Geometry: final body of the model. Coordinates: model frame, mm. A direction names the side the tool comes from. Round coordinates to 2 decimals unless told otherwise and drop trailing zeros. Write each loop counter-clockwise with the first axis right and the second up, starting at its lowest first coordinate (ties: lowest second). Pieces come first, ordered by that corner, then holes. Notation, with made-up numbers: (34.5, 44.5) - (69.5, 44.5) arc R20 cw to (69.5, 51.5) - close; hole circle Ø9 at (37, -10). An arc over 180 degrees is marked (long way). Write each question's results on one line, items separated by ' | '.
from build123d import *
from build123d.topology import SkipClean

# Parameters (mm, degrees)
BASE_DISC_SKETCH_R         = 31
BASE_DISC_DEPTH            = 13
BASE_SLOT_SKETCH_3X_R      = 3
BASE_SLOTS_3X_DEPTH        = 6
CLAMP_START                = -24
CLAMP_LUG_DEPTH            = 24
LUG_HOLE_A_SKETCH_R        = 4.680098696
LUG_HOLE_A_DEPTH           = 57.727418415
LUG_HOLE_B_SKETCH_R        = 5.830404683
LUG_HOLE_B_DEPTH           = 59.693575035
CLAMP_LUG_PATTERN_3X_COUNT = 3
FACE_RECESS_SKETCH_R       = 10
FACE_RECESS_2MM_DEPTH      = 2
LUG_CHAMFER_5MM_SIZE       = 5


with BuildPart() as part:
    # Base Disc Sketch → Base Disc (new body)
    with BuildSketch(Plane.XY):
        with Locations(Location((0, 0, 0), (0, 0, 180))):
            Circle(BASE_DISC_SKETCH_R)
    extrude(amount=BASE_DISC_DEPTH)

    # Base Slot Sketch 3x → Base Slots 3x (cut)
    with BuildSketch(Plane.XY):
        with Locations((-6.470476128, -24.148145657)):
            Circle(BASE_SLOT_SKETCH_3X_R)
        with Locations((-17.67766953, 17.67766953)):
            Circle(BASE_SLOT_SKETCH_3X_R)
        with Locations((24.148145657, 6.470476128)):
            Circle(BASE_SLOT_SKETCH_3X_R)
    extrude(amount=BASE_SLOTS_3X_DEPTH, mode=Mode.SUBTRACT)

    # Clamp Lug Sketch → Clamp Lug (add)
    with SkipClean():  # the faces are left unmerged after this step: merging them gives an invalid solid
        with BuildSketch(Plane.XY.offset(CLAMP_START)):
            with BuildLine():
                Line((5, 8.660254038), (5, 30.594117082))
                ThreePointArc((5, 30.594117082), (7.526051267, 30.072554802), (10, 29.342801502))
                Line((10, 29.342801502), (10, 8.306623863))
                ThreePointArc((10, 8.306623863), (10.309933784, 5.952443046), (12.193747285, 4.506942106))
                Line((12.193747285, 4.506942106), (30.411611519, -6.011146713))
                ThreePointArc((30.411611519, -6.011146713), (29.806622049, -8.518525814), (28.995282599, -10.966931522))
                Line((28.995282599, -10.966931522), (10, 0))
                ThreePointArc((10, 0), (8.660254038, 5), (5, 8.660254038))
            make_face()
        clamp_lug = extrude(amount=CLAMP_LUG_DEPTH)

    # Lug Hole A Sketch → Lug Hole A (cut, through all)
    with SkipClean():  # the faces are left unmerged after this step: merging them gives an invalid solid
        with BuildSketch(Plane(origin=(10, 0, 0), x_dir=(0, 0, -1), z_dir=(1, 0, 0))):
            with Locations(Location((14, 19.342801502, 0), (0, 0, 90))):
                Circle(LUG_HOLE_A_SKETCH_R)
        lug_hole_a = extrude(amount=-LUG_HOLE_A_DEPTH, mode=Mode.SUBTRACT)

    # Lug Hole B Sketch → Lug Hole B (cut, through all)
    with SkipClean():  # the faces are left unmerged after this step: merging them gives an invalid solid
        with BuildSketch(Plane(origin=(5, 8.660254038, 0), x_dir=(0.8660254037844388, -0.4999999999999998, 0), z_dir=(0.4999999999999998, 0.8660254037844388, 0))):
            with Locations(Location((19.342801502, 14, 0), (0, 0, 180))):
                Circle(LUG_HOLE_B_SKETCH_R)
        lug_hole_b = extrude(amount=-LUG_HOLE_B_DEPTH, mode=Mode.SUBTRACT)

    # Clamp Lug Pattern 3x: Clamp Lug, Lug Hole A, Lug Hole B ×3 about axis
    with SkipClean():  # the faces are left unmerged after this step: merging them gives an invalid solid
        clamp_lug_pattern_3x_axis = Axis((0, 0, 0), (0, 0, 1))
        add([clamp_lug.rotate(clamp_lug_pattern_3x_axis, i * 360 / CLAMP_LUG_PATTERN_3X_COUNT) for i in range(1, CLAMP_LUG_PATTERN_3X_COUNT)])
        add([lug_hole_a.rotate(clamp_lug_pattern_3x_axis, i * 360 / CLAMP_LUG_PATTERN_3X_COUNT) for i in range(1, CLAMP_LUG_PATTERN_3X_COUNT)], mode=Mode.SUBTRACT)
        add([lug_hole_b.rotate(clamp_lug_pattern_3x_axis, i * 360 / CLAMP_LUG_PATTERN_3X_COUNT) for i in range(1, CLAMP_LUG_PATTERN_3X_COUNT)], mode=Mode.SUBTRACT)

    # Face Recess Sketch → Face Recess 2mm (cut)
    with SkipClean():  # the faces are left unmerged after this step: merging them gives an invalid solid
        with BuildSketch(Plane(origin=(0, 0, 0), x_dir=(-1, 0, 0), z_dir=(0, 0, -1))):
            Circle(FACE_RECESS_SKETCH_R)
        extrude(amount=-FACE_RECESS_2MM_DEPTH, mode=Mode.SUBTRACT)

    # Lug Chamfer 5mm
    lug_chamfer_5mm_edges = [part.edges().sort_by_distance(p)[0] for p in [
        (7.526051267, 30.072554802, -24),
        (29.806622049, -8.518525814, -24),
        (-29.806622049, -8.518525814, -24),
        (-7.526051267, 30.072554802, -24),
        (22.280570782, -21.554028988, -24),
        (-22.280570782, -21.554028988, -24),
    ]]
    chamfer(lug_chamfer_5mm_edges, length=LUG_CHAMFER_5MM_SIZE)


solid = part.part
Q1. Section query B-B, the plane x = 0. Return loops of the section in (y, z).
Answer block:
outline: (-31, 0) - (-11.9, 0) - (-11.9, -24) - (-10, -24) - (-10, 2) - (10, 2) - (10, 0) - (31, 0) - (31, 13) - (-31, 13) - close
Q2. Pin query (flat end, axial travel): pin 1 (21.5 mm diameter, centred on x = -17.5, y = -5, fed in from -Z); pin 2 (6.5 mm diameter, centred on x = -21, y = 18.5, fed in from -Z); pin 3 (4 mm diameter, centred on y = -7.5, z = -19, fed in from -X); pin 4 (1.5 mm diameter, centred on x = 5, z = -17, fed in from -Y). Return the tip coordinate at first contact, or that it passes through.
Answer block:
pin 1: z = -24 | pin 2: z = 0 | pin 3: x = -30.41 | pin 4: y = -14.87
Q3. Access query for faces 1 (the flat face through (-21.43, -0.826, -6.835)), 2 (the flat face through (9.41, -16.98, -9.5)), 3 (the cylindrical face through (-17.769, -1.639, -9.084)), 4 (the flat face through (-5, 20, -7)), 5 (the cylindrical face through (-20.058, 15.852, 2.958)). Directions: +Z, -Z, +X, -X, +Y, -Y. A direction counts if a zero-diameter tool reaches every point of the face in a straight line with its end or side. Return the directions, or none.
Answer block:
face 1: -Z, -X, +Y | face 2: -Z, -Y | face 3: none | face 4: -Z, +Y | face 5: -Z
Q4. Section query C-C, the plane y = 16.5. Return loops of the section in (x, z), plus the area to 3 significant figures.
Answer block:
outline: (-26.24, 0) - (-20.44, 0) - (-20.44, 6) - (-14.92, 6) - (-14.92, 0) - (-10, 0) - (-10, -8.91) - (-5, -8.91) - (-5, 0) - (5, 0) - (5, -8.91) - (10, -8.91) - (10, 0) - (26.24, 0) - (26.24, 13) - (-26.24, 13) - close; (-10, -24) - (-5, -24) - (-5, -19.09) - (-10, -19.09) - close; (5, -24) - (10, -24) - (10, -19.09) - (5, -19.09) - close | area: 787 mm2
Q5. Ray query, line 1 along X through (y, z) = (14, -10.5); line 2 along Y through (x, z) = (-10.5, -6); line 3 along Z through (x, y) = (-18.5, 9.5). Return the intervals inside material, ascending.
Answer block:
line 1: -10 to -5, 5 to 10 | line 2: -17.61 to -11.84, -0.29 to 5.66 | line 3: 0 to 13
Q6. Section query A-A, the plane z = -5.5. Return loops of the section in (x, y).
Answer block:
outline: (-30.41, -6.01) arc R31 ccw to (-29, -10.97) - (-10, 0) arc R10 cw to (-5, 8.66) - (-5, 30.59) arc R31 ccw to (-10, 29.34) - (-10, 8.31) arc R3.1 cw to (-12.19, 4.51) - close; (-24, -19.63) arc R31 ccw to (-20.41, -23.33) - (-2.19, -12.81) arc R3.1 cw to (2.19, -12.81) - (20.41, -23.33) arc R31 ccw to (24, -19.63) - (5, -8.66) arc R10 cw to (-5, -8.66) - close; (5, 8.66) arc R10 cw to (10, 0) - (29, -10.97) arc R31 ccw to (30.41, -6.01) - (12.19, 4.51) arc R3.1 cw to (10, 8.31) - (10, 29.34) arc R31 ccw to (5, 30.59) - close
Q7. Mould query, pull axis Y, two halves, no side actions, for faces 6 (the cylindrical face through (7.465, 16.208, -9.084)), 7 (the flat face through (21.18, -0.68, -6.83)), 8 (the conical face through (-19.8, -20.5, -21.5)), 9 (the flat face through (-19.365, -5.407, -6.835)). Classes: pulls with the +Y half, pulls with the -Y half, needs draft (parallel to the pull), parting line crosses it, or undercut.
Answer block:
face 6: undercut | face 7: pulls with the +Y half | face 8: pulls with the -Y half | face 9: undercut
Q8. Section query D-D, the plane z = 1. Return loops of the section in (x, y).
Answer block:
outline: circle Ø62 at (0, 0); hole circle Ø6 at (-17.68, 17.68); hole circle Ø20 at (0, 0); hole circle Ø6 at (-6.47, -24.15); hole circle Ø6 at (24.15, 6.47)
